```python
from build123d import *

# Parameters (mm, degrees)
BOSS_EXTRUDE_1_DEPTH = 20
BOSS_EXTRUDE_2_DEPTH = 20
SKETCH_3_R           = 45
BOSS_EXTRUDE_3_DEPTH = 37


with BuildPart() as part:
    # Sketch 1 → Boss-Extrude 1 (new body)
    with BuildSketch(Plane(origin=(0, 0, 0), x_dir=(1, 0, 0), z_dir=(0, 1, 0))):
        with BuildLine():
            Line((48, 90), (-48, 90))
            ThreePointArc((-48, 90), (-56.485281374, 86.485281374), (-60, 78))
            Line((-60, 78), (-60, -78))
            ThreePointArc((-60, -78), (-56.485281374, -86.485281374), (-48, -90))
            Line((-48, -90), (48, -90))
            ThreePointArc((48, -90), (56.485281374, -86.485281374), (60, -78))
            Line((60, -78), (60, 78))
            ThreePointArc((60, 78), (56.485281374, 86.485281374), (48, 90))
        make_face()
    extrude(amount=BOSS_EXTRUDE_1_DEPTH)

    # Sketch 2 → Boss-Extrude 2 (add)
    with BuildSketch(Plane.XZ):
        with BuildLine():
            Line((-48, -80), (48, -80))
            ThreePointArc((48, -80), (49.414213562, -79.414213562), (50, -78))
            Line((50, -78), (50, 78))
            ThreePointArc((50, 78), (49.414213562, 79.414213562), (48, 80))
            Line((48, 80), (-48, 80))
            ThreePointArc((-48, 80), (-49.414213562, 79.414213562), (-50, 78))
            Line((-50, 78), (-50, -78))
            ThreePointArc((-50, -78), (-49.414213562, -79.414213562), (-48, -80))
        make_face()
    extrude(amount=BOSS_EXTRUDE_2_DEPTH)

    # Sketch 3 → Boss-Extrude 3 (add, symmetric)
    with BuildSketch(Plane(origin=(0, 0, 0), x_dir=(0, 0, -1), z_dir=(1, 0, 0))):
        with BuildLine():
            Line((-74.74949799, 206.124748995), (-90, 20))
            Line((-90, 20), (90, 20))
            Line((90, 20), (74.74949799, 206.124748995))
            ThreePointArc((74.74949799, 206.124748995), (0, 275), (-74.74949799, 206.124748995))
        make_face()
        with Locations((0, 200)):
            Circle(SKETCH_3_R, mode=Mode.SUBTRACT)
    extrude(amount=BOSS_EXTRUDE_3_DEPTH, both=True)


solid = part.part
```
Work out the finished part from the listing and answer in its coordinate system (mm). A direction names the side the tool comes from. Coordinates: 2 decimals unless noted, no trailing zeros. Write each loop counter-clockwise with the first axis right and the second up, starting at its lowest first coordinate (ties: lowest second). Pieces come first, ordered by that corner, then holes. Notation, with made-up numbers: (-13, 27.25) - (36, 27.25) arc R27 ccw to (36, 48.25) - close; hole circle Ø1 at (24, -2). An arc over 180 degrees is marked (long way). Answer as a JSON object with one key per item and string values.
Q1. Find section D-D (x = -40.5). Write down the section's boundary in (y, z).
Results list:
{"outline": "(-20, -80) - (0, -80) - (0, -90) - (20, -90) - (20, 90) - (0, 90) - (0, 80) - (-20, 80) - close"}
Q2. Which of the six approach directions +Z, -Z, +X, -X, +Y, -Y give full straight-line access (tool end or side, diameter ignored) to faces 1 (the flat face through (-1, -10, -80)), 2 (the flat face through (37, 121, 1)), 3 (the flat face through (-54, 0, -14)), 4 (the flat face through (-49, 20, -1)), 5 (the flat face through (-50, -10, 1))?
Results list:
{"face 1": "-Z, +X, -X, -Y", "face 2": "+Z, -Z, +X, +Y", "face 3": "-Y", "face 4": "+Z, -Z, -X, +Y", "face 5": "+Z, -Z, -X, -Y"}
Q3. Find section A-A (x = 18.5). Write down the section's boundary in (y, z), plus the area to 3 significant figures.
Results list:
{"outline": "(-20, -80) - (0, -80) - (0, -90) - (20, -90) - (206.12, -74.75) arc R75 ccw to (206.12, 74.75) - (20, 90) - (0, 90) - (0, 80) - (-20, 80) - close; hole circle Ø90 at (200, 0)", "area": "39,000 mm^2"}
Q4. Find section C-C (y = 200). Write down the section's boundary in (x, z).
Results list:
{"outline": "(-37, -75.25) - (37, -75.25) - (37, -45) - (-37, -45) - close; (-37, 45) - (37, 45) - (37, 75.25) - (-37, 75.25) - close"}
Q5. Find section B-B (z = -3). Write down the section's boundary in (x, y), plus the area to 3 significant figures.
Results list:
{"outline": "(-60, 0) - (-50, 0) - (-50, -20) - (50, -20) - (50, 0) - (60, 0) - (60, 20) - (37, 20) - (37, 155.1) - (-37, 155.1) - (-37, 20) - (-60, 20) - close; (-37, 244.9) - (37, 244.9) - (37, 274.94) - (-37, 274.94) - close", "area": "16,600 mm^2"}
Q6. For a pull along Z with two mould halves and no side action, classify faces 6 (the flat face through (1, -10, 80)), 7 (the cylindrical face through (-0.518, 237.944, -24.192)), 8 (the cylindrical face through (56.58, 9.86, -86.39)), 9 (the flat face through (-37, 121, 1)) as pulls with the +Z half, pulls with the -Z half, needs draft (parallel to the pull), parting line crosses it, or undercut.
Results list:
{"face 6": "pulls with the +Z half", "face 7": "undercut", "face 8": "pulls with the -Z half", "face 9": "needs draft"}
Q7. Given pin 1 Ø2 at (y, z) = (163.5, 41.5) entering from +X; pin 2 Ø6 at (x, y) = (13, -8.5) entering from +Z; pin 3 Ø11.5 at (x, z) = (49, 7.5) entering from +Y, each flat-ended and moving along its own axis, determine where each tip first touches the part or whether it passes through.
Results list:
{"pin 1": "stops at x = 37", "pin 2": "stops at z = 80", "pin 3": "stops at y = 20"}
Q8. Consider L1, parallel to Y at x = 8, z = 0; L2, parallel to Y at x = 46, z = 58; L3, parallel to X at y = 99, z = -57.5. Determine where each line is inside the solid, lowest interval first. Write a range as from..to.
Results list:
{"L1": "y = -20..155, 245..275", "L2": "y = -20..20", "L3": "x = -37..37"}
